For this review, take the finished solid that the model builds, in its own axes (mm). Give positions to 0.01 mm unless a question says otherwise; leave off trailing zeros. Write each loop counter-clockwise with the first axis right and the second up, starting at its lowest first coordinate (ties: lowest second). Pieces come first, ordered by that corner, then holes.
1) We need section A-A on x = -10. Give the boundary of the cut face in (y, z), and give its area (3 significant figures).
2) We need section B-B on z = -32.5. Give the boundary of the cut face in (x, y).
3) We need section C-C on x = -0.25. Give the boundary of the cut face in (y, z), and give its area (3 significant figures).
4) For P1, Ø1.5, axis at x = -8.5, z = -34.5, coming from the +Y side, flat-tipped, find the tip position at first contact; note if it passes through.
5) Wall thickness on line 1 along Y through (x, z) = (-7.5, -13.5); line 2 along Y through (x, z) = (-9, -19): over which ranges is each line inside the solid? List them lowest first.
from build123d import *

# Parameters (mm, degrees)
SKETCH2_W           = 25
SKETCH2_H           = 126
BOSS_EXTRUDE1_DEPTH = 80
CHAMFER1_SIZE       = 15


with BuildPart() as part:
    # Sketch2 → Boss-Extrude1 (new, symmetric)
    with BuildSketch(Plane(origin=(0, 0, 0), x_dir=(1, 0, 0), z_dir=(0, 1, 0))):
        Rectangle(SKETCH2_W, SKETCH2_H)
    extrude(amount=BOSS_EXTRUDE1_DEPTH, both=True)

    # Chamfer1
    chamfer1_edges = [part.edges().sort_by_distance(p)[0] for p in [
        (-12.5, 80, 0),
    ]]
    chamfer(chamfer1_edges, length=CHAMFER1_SIZE)


solid = part.part
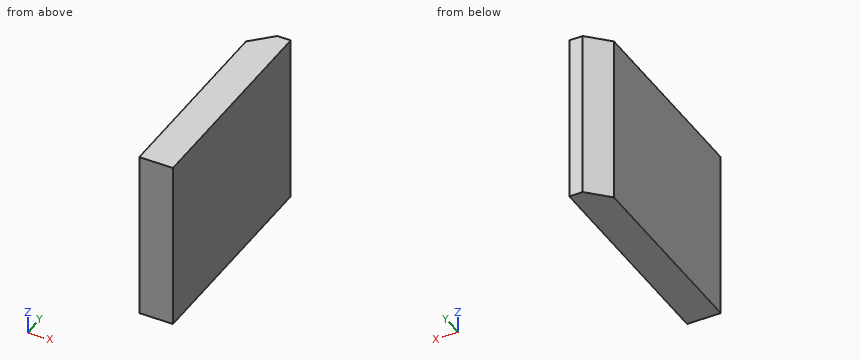
Results list:
1. outline: (-80, -63) - (67.5, -63) - (67.5, 63) - (-80, 63) - close
1. area: 18,600 mm2
2. outline: (-12.5, -80) - (12.5, -80) - (12.5, 80) - (2.5, 80) - (-12.5, 65) - close
3. outline: (-80, -63) - (77.25, -63) - (77.25, 63) - (-80, 63) - close
3. area: 19,800 mm2
4. P1: stops at y = 69.75
5. line 1: y = -80 to 70
5. line 2: y = -80 to 68.5
